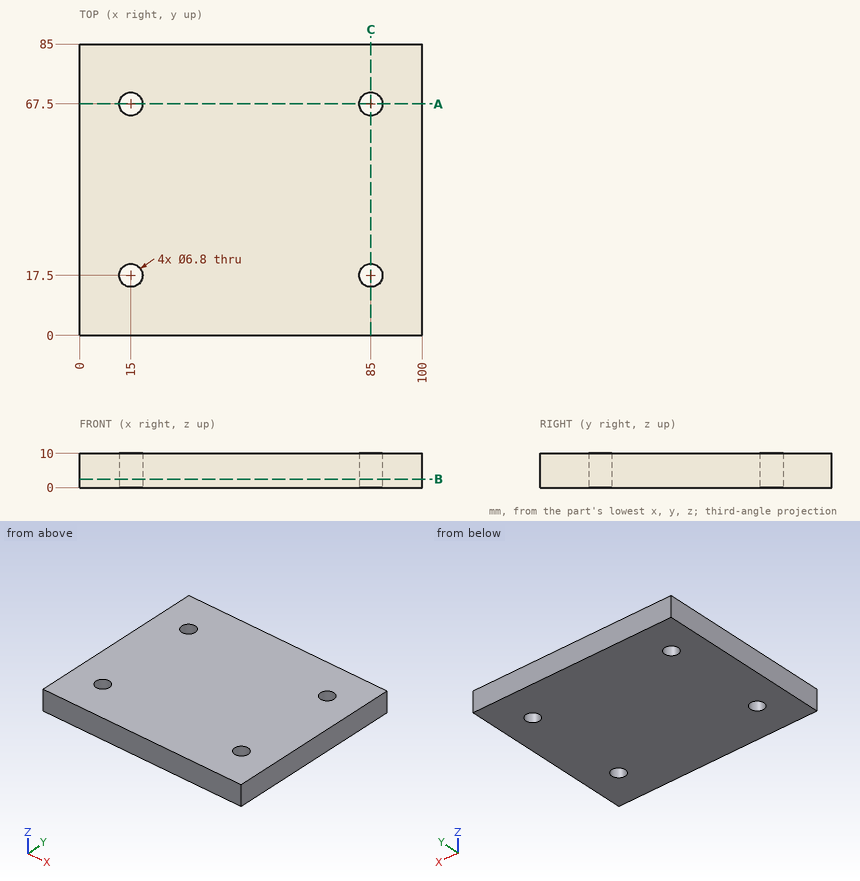
Can you work these out from the drawing? Everything is in mm from the part's minimum corner. Round coordinates to 2 decimals unless told otherwise and drop trailing zeros. Order: outer loops, then holes, each group sorted by start corner. A loop starts at its lowest first (then second) coordinate and runs counter-clockwise, first axis right, second up.
(1) If I drill on L1, parallel to Y at x = 85, z = 6.5; L2, parallel to X at y = 15.5, z = 3.25, over which ranges is the centre line in solid material (lowest first)?
Results are:
L1: y = 0 to 14.1, 20.9 to 64.1, 70.9 to 85
L2: x = 0 to 12.25, 17.75 to 82.25, 87.75 to 100
(2) If we section it at B-B (z = 2.5): Please give me the cut outline in (x, y).
Results are:
outline: (0, 0) - (100, 0) - (100, 85) - (0, 85) - close; hole circle Ø6.8 at (15, 17.5); hole circle Ø6.8 at (15, 67.5); hole circle Ø6.8 at (85, 17.5); hole circle Ø6.8 at (85, 67.5)
(3) If we section it at A-A (y = 67.5): Please give me the cut outline in (x, z), plus the area to 3 significant figures.
Results are:
outline: (0, 0) - (11.6, 0) - (11.6, 10) - (0, 10) - close; (18.4, 0) - (81.6, 0) - (81.6, 10) - (18.4, 10) - close; (88.4, 0) - (100, 0) - (100, 10) - (88.4, 10) - close
area: 864 mm2
(4) If we section it at C-C (x = 85): Please give me the cut outline in (y, z).
Results are:
outline: (0, 0) - (14.1, 0) - (14.1, 10) - (0, 10) - close; (20.9, 0) - (64.1, 0) - (64.1, 10) - (20.9, 10) - close; (70.9, 0) - (85, 0) - (85, 10) - (70.9, 10) - close
